Check sheet for the modelled part. Datum: model origin and axes. Units: mm. Give positions to 0.01 mm unless a question says otherwise; leave off trailing zeros. Order: outer loops, then holes, each group sorted by start corner. A loop starts at its lowest first (then second) coordinate and runs counter-clockwise, first axis right, second up.
```python
from build123d import *

# Parameters (mm, degrees)
SKETCH_1_R             = 3
EXTRUDE_1_DEPTH        = 45
HOLE_WIZARD_M3_1_D     = 2.5
HOLE_WIZARD_M3_1_DEPTH = 7.5
HOLE_WIZARD_M3_1_TIP   = 0.751075774
CHAMFER_1_SIZE         = 0.5


with BuildPart() as part:
    # 草图1 → 凸台-拉伸1 (new body)
    with BuildSketch(Plane.XY):
        with Locations(Location((0, 0, 0), (0, 0, 180))):
            Circle(SKETCH_1_R)
    extrude(amount=EXTRUDE_1_DEPTH)

    # M3 螺纹孔1
    with Locations(Plane(origin=(0, 0, 0), x_dir=(-1, 0, 0), z_dir=(0, 0, -1))):
        with Locations((0, 0)):
            Hole(HOLE_WIZARD_M3_1_D / 2, depth=HOLE_WIZARD_M3_1_DEPTH)
            with Locations((0, 0, -(HOLE_WIZARD_M3_1_DEPTH + HOLE_WIZARD_M3_1_TIP / 2))):  # 118° drill point
                Cone(0, HOLE_WIZARD_M3_1_D / 2, HOLE_WIZARD_M3_1_TIP, mode=Mode.SUBTRACT)

    # 倒角1
    chamfer_1_edges = [part.edges().sort_by_distance(p)[0] for p in [
        (3, 0, 0),
        (3, 0, 45),
    ]]
    chamfer(chamfer_1_edges, length=CHAMFER_1_SIZE)


solid = part.part
```
Q1. Go/stop test with flat-tipped pins: P1, Ø1.5, axis at y = -2.5, z = 38, coming from the +X side; P2, Ø1.5, axis at x = -1, z = 34, coming from the +Y side. Record where each tip stops, or that it passes through.
Q2. Draft check along Y on faces 1 (the conical face through (0.05, -0.21, 8.12)), 2 (the cylindrical face through (-0.27, -1.22, 3.8)), 3 (the cylindrical face through (-2.86, -0.9, 22.19)), 4 (the flat face through (0, 0, 45)). Enter one of: pulls with the +Y half, pulls with the -Y half, needs draft (parallel to the pull), parting line crosses it, or undercut.
Q3. Sectioned sample at A-A, the plane z = 39.5. Record the cut outline in (x, y).
Q4. Material ranges on line 1 (Y direction, x = 0, z = 4.5); line 2 (X direction, y = -0.2, z = 42.5); line 3 (Y direction, x = 1.65, z = 12), recorded low to high.
Filled in:
1. P1: stops at x = 2.44
1. P2: stops at y = 2.99
2. face 1: undercut
2. face 2: undercut
2. face 3: parting line crosses it
2. face 4: needs draft
3. outline: circle Ø6 at (0, 0)
4. line 1: y = -3 to -1.25, 1.25 to 3
4. line 2: x = -2.99 to 2.99
4. line 3: y = -2.51 to 2.51
